Read the model definition and answer for the solid it produces. Units are mm, in the model's axes. A direction names the side the tool comes from. Coordinates: 2 decimals unless noted, no trailing zeros. Write each loop counter-clockwise with the first axis right and the second up, starting at its lowest first coordinate (ties: lowest second). Pieces come first, ordered by that corner, then holes.
Item 1: This flat-tipped pin is pushed along its axis until it touches: P1, Ø3, axis at x = 63, z = 0, coming from the +Y side. Where does it stop, or does it pass through?
Item 2: Section A-A (x = 11) is taken. Give the vertices of the cut face in (y, z), then the cut area to 3 significant figures.
Item 3: Straight lines are drawn through the part: probe 1 along X at (y, z) = (2.75, 0); probe 2 along X at (y, z) = (7.2, 0); probe 3 along Z at (x, y) = (41.5, 1). For each, find the intervals that lie inside material, in ascending order.
Item 4: Section B-B (z = 0) is taken. Give the vertices of the cut face in (x, y).
Item 5: Section C-C (y = 2.75) is taken. Give the vertices of the cut face in (x, z).
Item 6: A tool of negligible diameter and unlimited length cuts with its end or side. For faces 1 (the face through (64.686, 7.014, 1.075)), 2 (the face through (53.874, 3.944, -4.972)), 3 (the face through (22, 4, -2.3)), from which of +Z, -Z, +X, -X, +Y, -Y can it reach the whole face along a straight path? Write none if from no direction.
Item 7: Determine the mould class of faces 4 (the face through (22, 4, -6)), 5 (the face through (66.913, 3.944, -0.086)), 6 (the face through (62, 6, 1)), 7 (the face through (54.126, 3.944, 4.943)) for opening direction Z: released by +Z, released by -Z, zero draft, split by the parting line, or undercut.
from build123d import *

# Parameters (mm, degrees)
BOSS_EXTRUDE1_DEPTH = 8
SKETCH2_R           = 2
CUT_EXTRUDE1_DEPTH  = 2
SKETCH3_R           = 1
CUT_EXTRUDE2_DEPTH  = 68.657428272


with BuildPart() as part:
    # Sketch1 → Boss-Extrude1 (new body)
    with BuildSketch(Plane(origin=(0, 0, 0), x_dir=(1, 0, 0), z_dir=(0, 1, 0))):
        with BuildLine():
            Line((0, 6), (45, 6))
            Line((45, 6), (63, 3.914330307))
            ThreePointArc((63, 3.914330307), (66.914330307, 0), (63, -3.914330307))
            Line((63, -3.914330307), (45, -6))
            Line((45, -6), (0, -6))
            ThreePointArc((0, -6), (-6, 0), (0, 6))
        make_face()
        with BuildLine():
            Line((0, 2.3), (45, 2.3))
            ThreePointArc((45, 2.3), (47.3, 0), (45, -2.3))
            Line((45, -2.3), (0, -2.3))
            ThreePointArc((0, -2.3), (-2.3, 0), (0, 2.3))
        make_face(mode=Mode.SUBTRACT)
    extrude(amount=BOSS_EXTRUDE1_DEPTH)

    # Sketch2 → Cut-Extrude1 (cut)
    with BuildSketch(Plane(origin=(0, 8, 0), x_dir=(1, 0, 0), z_dir=(0, 1, 0))):
        with Locations(Location((63, 0, 0), (0, 0, 270))):
            Circle(SKETCH2_R)
    extrude(amount=-CUT_EXTRUDE1_DEPTH, mode=Mode.SUBTRACT)

    # Sketch3 → Cut-Extrude2 (cut, through all)
    with BuildSketch(Plane.XZ):
        with Locations(Location((63, 0, 0), (0, 0, 270))):
            Circle(SKETCH3_R)
    extrude(amount=-CUT_EXTRUDE2_DEPTH, mode=Mode.SUBTRACT)


solid = part.part
Established:
1. P1: stops at y = 6
2. outline: (0, -6) - (8, -6) - (8, -2.3) - (0, -2.3) - close; (0, 2.3) - (8, 2.3) - (8, 6) - (0, 6) - close
2. area: 59.2 mm2
3. probe 1: x = -6 to -2.3, 47.3 to 62, 64 to 66.91
3. probe 2: x = -6 to -2.3, 47.3 to 61, 65 to 66.91
3. probe 3: z = -6 to -2.3, 2.3 to 6
4. outline: (-6, 0) - (-2.3, 0) - (-2.3, 8) - (-6, 8) - close; (47.3, 0) - (62, 0) - (62, 6) - (61, 6) - (61, 8) - (47.3, 8) - close; (64, 0) - (66.91, 0) - (66.91, 8) - (65, 8) - (65, 6) - (64, 6) - close
5. outline: (0, -6) - (45, -6) - (63, -3.91) arc R3.91 ccw to (63, 3.91) - (45, 6) - (0, 6) arc R6 ccw to start; hole (0, -2.3) - (45, -2.3) arc R2.3 ccw to (45, 2.3) - (0, 2.3) arc R2.3 ccw to start; hole circle Ø2 at (63, 0)
6. face 1: +Y
6. face 2: -Z, +X, +Y, -Y
6. face 3: +Y, -Y
7. face 4: released by -Z
7. face 5: split by the parting line
7. face 6: undercut
7. face 7: released by +Z
